Can you work these out from the model? Positions are in its coordinate system, mm. Round coordinates to 2 decimals unless told otherwise and drop trailing zeros. Loops run counter-clockwise (first coordinate to the right, second up) from the corner with the lowest first, then second, coordinate; pieces in that order, holes last.
(1) I want a section at C-C on z = 109. Write out the boundary of the cut face in (x, y).
(2) If I drill on line 1 along Y through (x, z) = (0, 59); line 2 along Z through (x, y) = (-2.25, 7.25); line 3 along X through (y, z) = (-0.25, 42.5), over which ranges is the centre line in solid material (lowest first)?
(3) I want a section at A-A on y = 0. Write out the boundary of the cut face in (x, z), plus the area to 4 significant figures.
(4) Will these pins go through, and if not, where does the flat tip stop? pin 1 Ø8 at (x, z) = (3, 168.5) entering from -Y; pin 2 Ø6 at (y, z) = (-3.5, 25) entering from +X; pin 3 Ø2 at (x, y) = (-5.5, 6) entering from +Z.
from build123d import *

# Parameters (mm, degrees)
SKETCH_1_R      = 4.5
EXTRUDE_1_DEPTH = 15
SKETCH_2_R      = 6
EXTRUDE_2_DEPTH = 180
SKETCH_3_R      = 8
EXTRUDE_3_DEPTH = 5


with BuildPart() as part:
    # 草图1 → 凸台-拉伸1 (new body)
    with BuildSketch(Plane.XY):
        Circle(SKETCH_1_R)
    extrude(amount=EXTRUDE_1_DEPTH)

    # 草图2 → 凸台-拉伸2 (add)
    with BuildSketch(Plane.XY.offset(15)):
        with Locations(Location((0, 0, 0), (0, 0, 180))):
            Circle(SKETCH_2_R)
    extrude(amount=EXTRUDE_2_DEPTH)

    # 草图3 → 凸台-拉伸3 (add)
    with BuildSketch(Plane(origin=(0, 0, 15), x_dir=(-1, 0, 0), z_dir=(0, 0, -1))):
        Circle(SKETCH_3_R)
    extrude(amount=-EXTRUDE_3_DEPTH)


solid = part.part
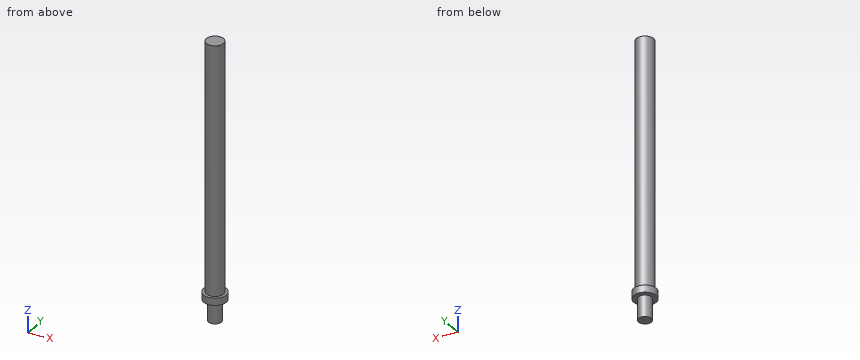
Filled sheet:
1. outline: circle Ø12 at (0, 0)
2. line 1: y = -6 to 6
2. line 2: z = 15 to 20
2. line 3: x = -5.99 to 5.99
3. outline: (-8, 15) - (-4.5, 15) - (-4.5, 0) - (4.5, 0) - (4.5, 15) - (8, 15) - (8, 20) - (6, 20) - (6, 195) - (-6, 195) - (-6, 20) - (-8, 20) - close
3. area: 2,315 mm2
4. pin 1: stops at y = -6
4. pin 2: stops at x = 5.98
4. pin 3: stops at z = 20
